Build history of the part. All positions in model axes, mm. A direction names the side the tool comes from. Round coordinates to 2 decimals unless told otherwise and drop trailing zeros. Order: outer loops, then holes, each group sorted by start corner. A loop starts at its lowest first (then second) coordinate and runs counter-clockwise, first axis right, second up. Notation, with made-up numbers: (27.25, 7) -> (85.25, 7) arc R19 ccw to (85.25, 34) -> close; hole circle Ø2 at (44.25, -2). An arc over 180 degrees is marked (long way). Answer as a JSON object with one key per item and string values.
from build123d import *

# Parameters (mm, degrees)
SKETCH_1_W      = 30
SKETCH_1_H      = 30
SKETCH_1_W_2    = 26
SKETCH_1_H_2    = 26
EXTRUDE_1_DEPTH = 1070


with BuildPart() as part:
    # 草图1 → 凸台-拉伸1 (new body)
    with BuildSketch(Plane.XY):
        Rectangle(SKETCH_1_W, SKETCH_1_H)
        Rectangle(SKETCH_1_W_2, SKETCH_1_H_2, mode=Mode.SUBTRACT)
    extrude(amount=EXTRUDE_1_DEPTH)


solid = part.part
1) Cut at C-C, the plane z = 940.5. Give the cut face in (x, y).
Checked values:
{"outline": "(-15, -15) -> (15, -15) -> (15, 15) -> (-15, 15) -> close; hole (-13, -13) -> (13, -13) -> (13, 13) -> (-13, 13) -> close"}
2) Probe L1, parallel to X at y = -3, z = 710. List the from-to ranges inside material, lowest first. Write a range as from..to.
Checked values:
{"L1": "x = -15..-13, 13..15"}
3) Which spindle directions (+Z, -Z, +X, -X, +Y, -Y) get a long thin tool onto all of the face, cutting with end or side? Do faces 1 (the face through (-15, 0, 528)), 2 (the face through (13, 0, 528)). Say none if no direction does.
Checked values:
{"face 1": "+Z, -Z, -X, +Y, -Y", "face 2": "+Z, -Z"}
4) Pull direction Y, two halves, no side cores. Call faces 3 (the face through (0, -15, 528)), 4 (the face through (-13, 0, 528)), 5 (the face through (0, 15, 528)): pulls with the +Y half, pulls with the -Y half, needs draft (parallel to the pull), parting line crosses it, or undercut.
Checked values:
{"face 3": "pulls with the -Y half", "face 4": "undercut", "face 5": "pulls with the +Y half"}
5) Cut at A-A, the plane x = 2.25. Give the cut face in (y, z), plus the area to 3 significant figures.
Checked values:
{"outline": "(-15, 0) -> (-13, 0) -> (-13, 1070) -> (-15, 1070) -> close; (13, 0) -> (15, 0) -> (15, 1070) -> (13, 1070) -> close", "area": "4,280 mm²"}
